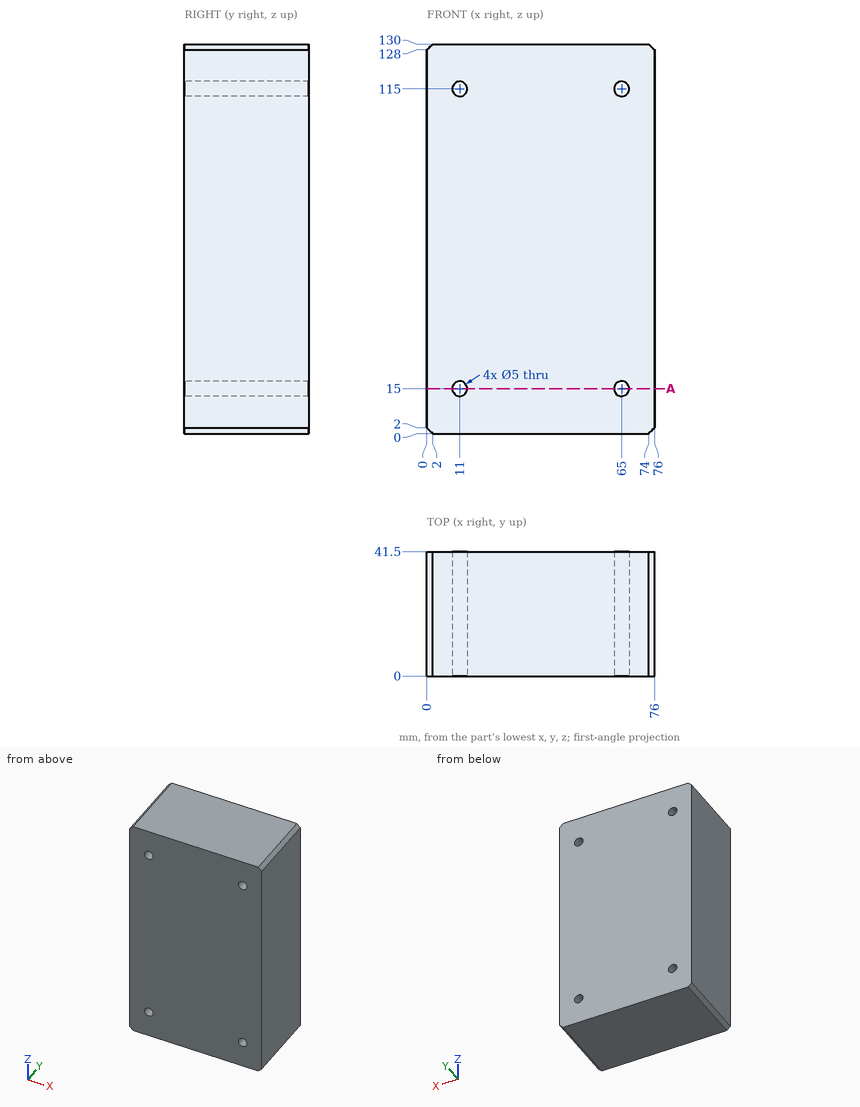
Design review of the part shown in the three views and the two pictorial views. Dimensions are in mm from the part's minimum x, y and z. Give positions to 0.01 mm unless a question says otherwise; leave off trailing zeros. Write each loop counter-clockwise with the first axis right and the second up, starting at its lowest first coordinate (ties: lowest second). Pieces come first, ordered by that corner, then holes. Notation, with made-up numbers: M -16.5,52 L -9.5,52 A18 ccw -9.5,59 Z; hole C 9.25,65.25 d6. An arc over 180 degrees is marked long. One line per item, written item: value.
1) Take a section at A-A, the plane z = 15. Write out the cut boundary in (x, y).
Results are:
outline: M 0,0 L 8.5,0 L 8.5,41.5 L 0,41.5 Z; M 13.5,0 L 62.5,0 L 62.5,41.5 L 13.5,41.5 Z; M 67.5,0 L 76,0 L 76,41.5 L 67.5,41.5 Z
2) For P1, Ø4.5, axis at x = 11, z = 115, coming from the -Y side, flat-tipped, find the tip position at first contact; note if it passes through.
Results are:
P1: passes through
3) For line 1 (X direction, y = 29, z = 115); line 2 (X direction, y = 29.5, z = 17); line 3 (Z direction, x = 13, y = 13.5), list the stretches that pass through material, from the lowest coordinate up. Write a range as from..to.
Results are:
line 1: x = 0..8.5, 13.5..62.5, 67.5..76
line 2: x = 0..9.5, 12.5..63.5, 66.5..76
line 3: z = 0..13.5, 16.5..113.5, 116.5..130
